```python
from build123d import *

# Parameters (mm, degrees)
BOSS_EXTRUDE1_DEPTH = 10
CHAMFER1_SIZE       = 10


with BuildPart() as part:
    # Sketch1 → Boss-Extrude1 (new body)
    with BuildSketch(Plane.XY):
        Polygon((0, 0), (-150, 0), (-150, -20), (-20, -100), (0, -100), align=None)
    extrude(amount=-BOSS_EXTRUDE1_DEPTH)

    # Chamfer1
    chamfer1_edges = [part.edges().sort_by_distance(p)[0] for p in [
        (0, 0, -5),
    ]]
    chamfer(chamfer1_edges, length=CHAMFER1_SIZE)


solid = part.part
```
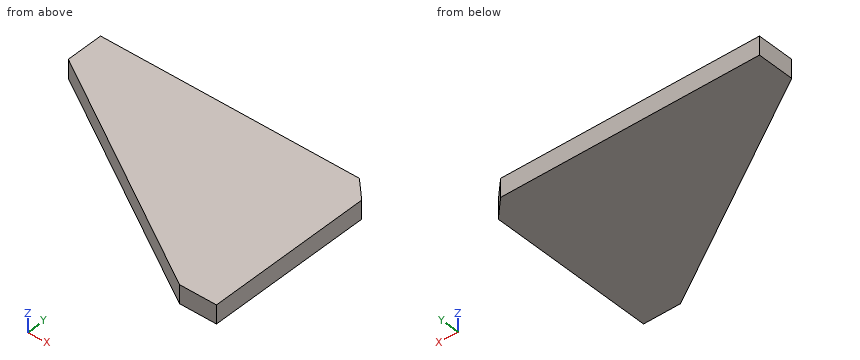
Can you work these out from the model? Positions are in its coordinate system, mm. Round coordinates to 2 decimals unless told otherwise and drop trailing zeros. Loops run counter-clockwise (first coordinate to the right, second up) from the corner with the lowest first, then second, coordinate; pieces in that order, holes last. Notation, with made-up numbers: M 58,82 L 74,82 A17 ccw 74,106 Z; hole C 16.5,66 d2. An arc over 180 degrees is marked long. Write item = value, one per line. Start each with the question number.
(1) Suppose I cut it at A-A on y = -90. Write out the boundary of the cut face in (x, z).
(2) I'm going to push flat-ended pins straight in: P1, Ø5, axis at y = -53.5, z = -3, coming from the -X side (3 decimals); P2, Ø2, axis at y = -62.5, z = -1.5, coming from the -X side. Where does each tip first touch, or does it pass through?
(3) Suppose I cut it at C-C on x = -65. Write out the boundary of the cut face in (y, z).
(4) I need wall thicknesses on line 1 along Y through (x, z) = (-66, -6.75); line 2 along X through (y, z) = (-36, -3); line 3 along X through (y, z) = (-79, -1.25) (3 decimals). Which ranges of each line are inside material? Lowest first, please.
(5) Suppose I cut it at B-B on z = -3. Write out the boundary of the cut face in (x, y), plus the area to 3 significant figures.
Answer block:
q1.outline = M -36.25,-10 L 0,-10 L 0,0 L -36.25,0 Z
q2.P1 = -99.625
q2.P2 = -82.56
q3.outline = M -72.31,-10 L 0,-10 L 0,0 L -72.31,0 Z
q4.line_1 = -71.69 to 0
q4.line_2 = -124 to 0
q4.line_3 = -54.125 to 0
q5.outline = M -150,-20 L -20,-100 L 0,-100 L 0,-10 L -10,0 L -150,0 Z
q5.area = 9,750 mm²
